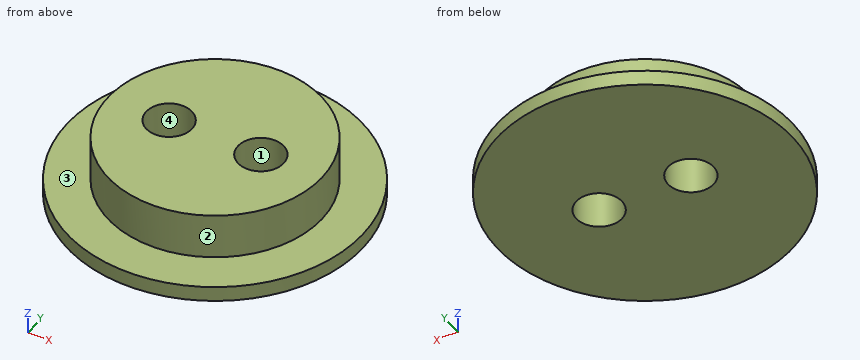
from build123d import *

# Parameters (mm, degrees)
SKETCH_1_R          = 29
EXTRUDE_1_DEPTH     = 3
SKETCH_2_R          = 21
EXTRUDE_2_DEPTH     = 9
SKETCH_3_R          = 4.5
CUT_EXTRUDE_1_DEPTH = 43.731721238


with BuildPart() as part:
    # 草图1 → 凸台-拉伸1 (new body)
    with BuildSketch(Plane.XY):
        Circle(SKETCH_1_R)
    extrude(amount=EXTRUDE_1_DEPTH)

    # 草图2 → 凸台-拉伸2 (add)
    with BuildSketch(Plane.XY.offset(3)):
        Circle(SKETCH_2_R)
    extrude(amount=EXTRUDE_2_DEPTH)

    # 草图3 → 切除-拉伸1 (cut, through all)
    with BuildSketch(Plane.XY.offset(12)):
        with Locations((-9, 0)):
            Circle(SKETCH_3_R)
        with Locations((9, 0)):
            Circle(SKETCH_3_R)
    extrude(amount=-CUT_EXTRUDE_1_DEPTH, mode=Mode.SUBTRACT)


solid = part.part
Geometry check sheet. Reference: the model listing, model coordinates, mm. Face numbers are marked on the shaded views. Coordinates: 2 decimals unless noted, no trailing zeros. Write each loop counter-clockwise with the first axis right and the second up, starting at its lowest first coordinate (ties: lowest second). Pieces come first, ordered by that corner, then holes. Notation, with made-up numbers: (28.25, 56.25) -> (75.25, 56.25) arc R18 ccw to (75.25, 86.25) -> close; hole circle Ø10 at (62, 29.25). An arc over 180 degrees is marked (long way). One line per question, with ' | ' between items.
1. Draft check along X on the marked faces 1, 2, 3 and 4. Enter one of: +X half, -X half, draft (parallel to the pull), parting line (faces both ways), or undercut.
Answers:
face 1: undercut | face 2: parting line | face 3: draft | face 4: undercut
2. Thickness scan on probe 1 along X at (y, z) = (-4, 4); probe 2 along Z at (x, y) = (15, 18.5); probe 3 along Y at (x, z) = (9, 8.75). Record the ranges inside material, lowest first. Write a range as from..to.
Answers:
probe 1: x = -20.62..-11.06, -6.94..6.94, 11.06..20.62 | probe 2: z = 0..3 | probe 3: y = -18.97..-4.5, 4.5..18.97
3. Cross-section at A-A on y = 0. Record the cut outline in (x, z), and give its area (3 significant figures).
Answers:
outline: (-29, 0) -> (-13.5, 0) -> (-13.5, 12) -> (-21, 12) -> (-21, 3) -> (-29, 3) -> close; (-4.5, 0) -> (4.5, 0) -> (4.5, 12) -> (-4.5, 12) -> close; (13.5, 0) -> (29, 0) -> (29, 3) -> (21, 3) -> (21, 12) -> (13.5, 12) -> close | area: 336 mm²
4. Cross-section at C-C on z = 7.75. Record the cut outline in (x, y), and give its area (3 significant figures).
Answers:
outline: circle Ø42 at (0, 0); hole circle Ø9 at (-9, 0); hole circle Ø9 at (9, 0) | area: 1,260 mm²
5. Depth check by flat-ended pin: pin 1 Ø6 at (y, z) = (-12.5, 3.5) entering from -X; pin 2 Ø5 at (x, z) = (12, 10) entering from +Y; pin 3 Ø2 at (x, z) = (-7.5, 5.5) entering from +Y. Enter the tip coordinate at first touch or a pass-through.
Answers:
pin 1: stops at x = -27.39 | pin 2: stops at y = 18.73 | pin 3: stops at y = 19.97
6. Cross-section at D-D on x = 0. Record the cut outline in (y, z).
Answers:
outline: (-29, 0) -> (29, 0) -> (29, 3) -> (21, 3) -> (21, 12) -> (-21, 12) -> (-21, 3) -> (-29, 3) -> close
7. Cross-section at B-B on x = 9. Record the cut outline in (y, z), and give its area (3 significant figures).
Answers:
outline: (-27.57, 0) -> (-4.5, 0) -> (-4.5, 12) -> (-18.97, 12) -> (-18.97, 3) -> (-27.57, 3) -> close; (4.5, 0) -> (27.57, 0) -> (27.57, 3) -> (18.97, 3) -> (18.97, 12) -> (4.5, 12) -> close | area: 399 mm²
